Source: three-view drawing plus pictorial views. Frame: mm from the lowest corner of the part. A direction names the side the tool comes from. Give positions to 0.01 mm unless a question says otherwise; leave off trailing zeros. Order: outer loops, then holes, each group sorted by start corner. A loop starts at its lowest first (then second) coordinate and runs counter-clockwise, first axis right, second up. Notation, with made-up numbers: (61, 23) -> (111, 23) arc R17 cw to (111, 48) -> close; hole circle Ø3 at (-1.75, 88). An arc over 180 degrees is marked (long way). One line per question, with ' | ' between items.
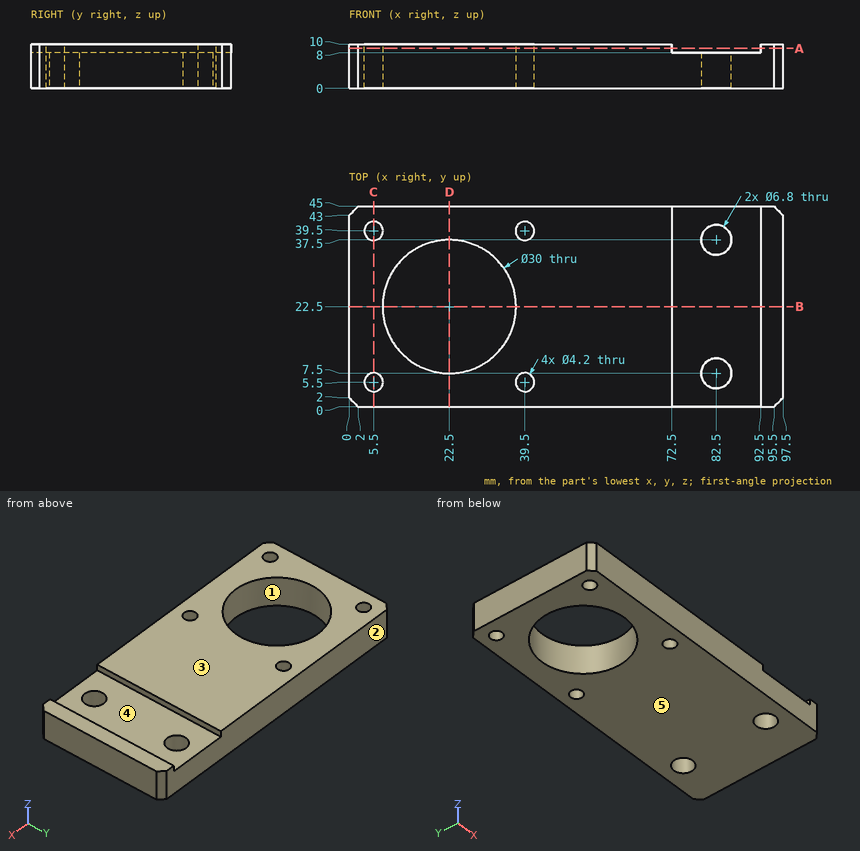
1) Material intervals for probe 1 along Y at (x, z) = (5.5, 2.25); probe 2 along Y at (x, z) = (82.5, 2.75); probe 3 along X at (y, z) = (6.5, 8.5), sorted ascending. Write a range as from..to.
Check result:
probe 1: y = 0..3.4, 7.6..37.4, 41.6..45 | probe 2: y = 0..4.1, 10.9..34.1, 40.9..45 | probe 3: x = 0..3.65, 7.35..37.65, 41.35..72.5, 92.5..97.5
2) Pull-direction query (Y, two-part tool) for the marked faces 1, 2 and 3; classes: +Y half, -Y half, draft (parallel to the pull), parting line (faces both ways), or undercut.
Check result:
face 1: undercut | face 2: +Y half | face 3: draft
3) Section A-A on z = 9. Return loops of the section in (x, y).
Check result:
outline: (0, 2) -> (2, 0) -> (72.5, 0) -> (72.5, 45) -> (2, 45) -> (0, 43) -> close; (92.5, 0) -> (95.5, 0) -> (97.5, 2) -> (97.5, 43) -> (95.5, 45) -> (92.5, 45) -> close; hole circle Ø4.2 at (5.5, 5.5); hole circle Ø4.2 at (5.5, 39.5); hole circle Ø30 at (22.5, 22.5); hole circle Ø4.2 at (39.5, 5.5); hole circle Ø4.2 at (39.5, 39.5)
4) Section B-B on y = 22.5. Return loops of the section in (x, z), plus the area to 3 significant figures.
Check result:
outline: (0, 0) -> (7.5, 0) -> (7.5, 10) -> (0, 10) -> close; (37.5, 0) -> (97.5, 0) -> (97.5, 10) -> (92.5, 10) -> (92.5, 8) -> (72.5, 8) -> (72.5, 10) -> (37.5, 10) -> close | area: 635 mm^2
5) Contact query for flat-ended pins moving along their axis: pin 1 Ø4 at (x, y) = (39.5, 5.5) entering from +Z; pin 2 Ø10 at (x, y) = (79, 25) entering from +Z. Output: stop coordinate, or through.
Check result:
pin 1: passes through | pin 2: stops at z = 8
6) Section C-C on x = 5.5. Return loops of the section in (y, z).
Check result:
outline: (0, 0) -> (3.4, 0) -> (3.4, 10) -> (0, 10) -> close; (7.6, 0) -> (37.4, 0) -> (37.4, 10) -> (7.6, 10) -> close; (41.6, 0) -> (45, 0) -> (45, 10) -> (41.6, 10) -> close
7) Section D-D on x = 22.5. Return loops of the section in (y, z).
Check result:
outline: (0, 0) -> (7.5, 0) -> (7.5, 10) -> (0, 10) -> close; (37.5, 0) -> (45, 0) -> (45, 10) -> (37.5, 10) -> close
8) Set-up query: the marked faces 4 and 5. Return all of +Z, -Z, +X, -X, +Y, -Y with unobstructed straight access to the full face (end or side cutting, diameter ignored); none if empty.
Check result:
face 4: +Z, +Y, -Y | face 5: -Z, +X, -X, +Y, -Y
